Part model, mm, in its own coordinate system. Face numbers are marked on the shaded views. A direction names the side the tool comes from. Coordinates: 2 decimals unless noted, no trailing zeros. Loops run counter-clockwise (first coordinate to the right, second up) from the corner with the lowest first, then second, coordinate; pieces in that order, holes last. Notation, with made-up numbers: M -13.5,-28 L 21.5,-28 A16 cw 21.5,-13 Z; hole C 68,72 d1. An arc over 180 degrees is marked long. Use CSV: the item, a comma, the result in double quotes. Start each with the question number.
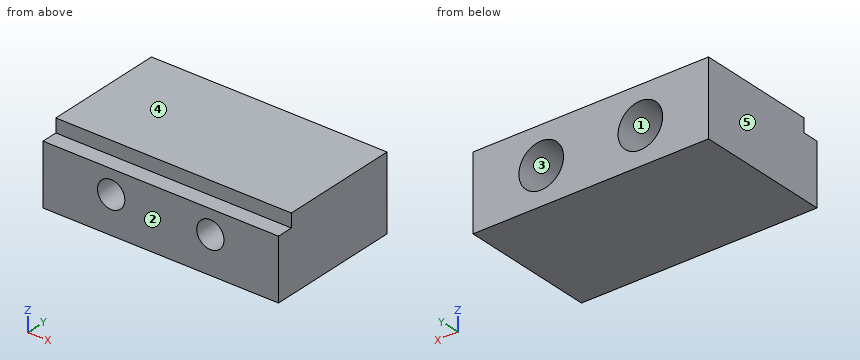
from build123d import *

# Parameters (mm, degrees)
SKETCH1_W           = 95
SKETCH1_H           = 30
BOSS_EXTRUDE1_DEPTH = 55
SKETCH2_R           = 5.5
CUT_EXTRUDE1_DEPTH  = 75.204110398
SKETCH3_R           = 9
CUT_EXTRUDE2_DEPTH  = 20
SKETCH4_W           = 5.5
SKETCH4_H           = 6.5
CUT_EXTRUDE3_DEPTH  = 172


with BuildPart() as part:
    # Sketch1 → Boss-Extrude1 (new body)
    with BuildSketch(Plane(origin=(0, 0, 0), x_dir=(1, 0, 0), z_dir=(0, 1, 0))):
        Rectangle(SKETCH1_W, SKETCH1_H)
    extrude(amount=BOSS_EXTRUDE1_DEPTH)

    # Sketch2 → Cut-Extrude1 (cut, through all)
    with BuildSketch(Plane(origin=(0, 55, 0), x_dir=(1, 0, 0), z_dir=(0, 1, 0))):
        with Locations(Location((-20, 0, 0), (0, 0, 270))):
            Circle(SKETCH2_R)
        with Locations(Location((20, 0, 0), (0, 0, 270))):
            Circle(SKETCH2_R)
    extrude(amount=-CUT_EXTRUDE1_DEPTH, mode=Mode.SUBTRACT)

    # Sketch3 → Cut-Extrude2 (cut)
    with BuildSketch(Plane(origin=(0, 55, 0), x_dir=(1, 0, 0), z_dir=(0, 1, 0))):
        with Locations(Location((-20, 0, 0), (0, 0, 270))):
            Circle(SKETCH3_R)
        with Locations(Location((20, 0, 0), (0, 0, 270))):
            Circle(SKETCH3_R)
    extrude(amount=-CUT_EXTRUDE2_DEPTH, mode=Mode.SUBTRACT)

    # Sketch4 → Cut-Extrude3 (cut)
    with BuildSketch(Plane.ZY.offset(47.5)):
        with Locations((12.25, 3.25)):
            Rectangle(SKETCH4_W, SKETCH4_H)
    extrude(amount=-CUT_EXTRUDE3_DEPTH, mode=Mode.SUBTRACT)


solid = part.part
1. Two-plate mould, pull along Z, no slides. Class the marked faces 3, 4 and 5: pulls with the +Z half, pulls with the -Z half, needs draft (parallel to the pull), parting line crosses it, or undercut.
2. Slice it at D-D, the plane x = 26.5. List the corners of the cut face in (y, z).
3. Slice it at C-C, the plane y = 32. List the corners of the cut face in (x, z).
4. Tool access for the marked faces 1 and 2: list every direction of +Z, -Z, +X, -X, +Y, -Y with a clear straight run to the whole face (end or side of a thin tool).
5. Pin check, flat tips, straight feed: pin 1 (5.5 mm diameter, centred on x = 15.5, z = -2.5, fed in from +Y); pin 2 (6 mm diameter, centred on x = 23.5, z = 13, fed in from -Y); pin 3 (2 mm diameter, centred on x = 13, y = 2, fed in from +Z). Stop position of each tip, or through.
6. Slice it at A-A, the plane z = 0. List the corners of the cut face in (x, y), and give its area (4 significant figures).
7. Wall check: probe 1 along X at (y, z) = (41.5, 0); probe 2 along Z at (x, y) = (-19.5, 19); probe 3 along Z at (x, y) = (20.5, 3.5). Give the ranges that are in metal, low to high.
8. Slice it at B-B, the plane x = -20. List the corners of the cut face in (y, z).
Found:
1,face 3,"undercut"
1,face 4,"pulls with the +Z half"
1,face 5,"needs draft"
2,outline,"M 0,-15 L 55,-15 L 55,-6.22 L 35,-6.22 L 35,6.22 L 55,6.22 L 55,15 L 6.5,15 L 6.5,9.5 L 0,9.5 Z"
3,outline,"M -47.5,-15 L 47.5,-15 L 47.5,15 L -47.5,15 Z; hole C -20,0 d11; hole C 20,0 d11"
4,face 1,"+Y"
4,face 2,"+Z, -Z, +X, -X, -Y"
5,pin 1,"y = 35"
5,pin 2,"y = 6.5"
5,pin 3,"z = 9.5"
6,outline,"M -47.5,0 L -25.5,0 L -25.5,35 L -29,35 L -29,55 L -47.5,55 Z; M -14.5,0 L 14.5,0 L 14.5,35 L 11,35 L 11,55 L -11,55 L -11,35 L -14.5,35 Z; M 25.5,0 L 47.5,0 L 47.5,55 L 29,55 L 29,35 L 25.5,35 Z"
6,area,"3,735 mm^2"
7,probe 1,"-47.5 to -29, -11 to 11, 29 to 47.5"
7,probe 2,"-15 to -5.48, 5.48 to 15"
7,probe 3,"-15 to -5.48, 5.48 to 9.5"
8,outline,"M 0,-15 L 55,-15 L 55,-9 L 35,-9 L 35,-5.5 L 0,-5.5 Z; M 0,5.5 L 35,5.5 L 35,9 L 55,9 L 55,15 L 6.5,15 L 6.5,9.5 L 0,9.5 Z"
